Can you work these out from the model? Positions are in its coordinate system, mm. A direction names the side the tool comes from. Give positions to 0.01 mm unless a question says otherwise; leave off trailing zeros. Loops run counter-clockwise (first coordinate to the right, second up) from the corner with the lowest first, then second, coordinate; pieces in that order, holes last. Notation, with made-up numbers: (18, 11) - (53, 11) arc R34 ccw to (53, 43) - close; hole circle Ø7 at (-34.5, 30.5). An arc over 180 degrees is marked (long way). Use a Markdown table: item, result. Add a question column.
```python
from build123d import *

# Parameters (mm, degrees)
BOSS_EXTRUDE1_DEPTH = 348
CUT_EXTRUDE1_DEPTH  = 350


with BuildPart() as part:
    # Sketch1 → Boss-Extrude1 (new body)
    with BuildSketch(Plane.XY):
        Polygon((0, 169.911519959), (-60, 139.911519959), (0, 109.911519959), (60, 139.911519959), align=None)
    extrude(amount=BOSS_EXTRUDE1_DEPTH)

    # Sketch2 → Cut-Extrude1 (cut)
    with BuildSketch(Plane.XY.offset(348)):
        Polygon((48.819660113, 139.911519959), (0, 164.321350015), (-48.819660113, 139.911519959), (0, 115.501689902), align=None)
    extrude(amount=-CUT_EXTRUDE1_DEPTH, mode=Mode.SUBTRACT)


solid = part.part
```
1. Suppose I cut it at A-A (z = 318). List the corners of the cut face in (x, y) for me, and give its area (3 significant figures).
2. Suppose I cut it at C-C (x = 41). List the corners of the cut face in (y, z) for me.
3. If we mould it in two halves opening along Y, with no side actions, what happens to faces 1 (the face through (24.752, 151.946, 176.436)), 2 (the face through (-14, 160, 348)), 3 (the face through (-30.42, 125.12, 171.56)), 4 (the face through (30.42, 154.7, 171.56))? For each: released by +Y, released by -Y, zero draft, split by the parting line, or undercut.
4. Please list where these lines run through material, in increasing order: line 1 along X through (y, z) = (140, 34.5); line 2 along Y through (x, z) = (34.5, 292.5); line 3 along X through (y, z) = (161, 243). Write a range as [from, to].
5. Suppose I cut it at B-B (y = 143.5). List the corners of the cut face in (x, z) for me, and give its area (3 significant figures).
6. Will these pins go through, and if not, where does the flat tip stop? P1, Ø12, axis at y = 159, z = 179.5, coming from the -X side; P2, Ø10, axis at x = 38, y = 148.5, coming from the -Z side; P3, Ø1, axis at x = -4, z = 56.5, coming from the +Y side; P4, Ø1.5, axis at x = -22, z = 226.5, coming from the -Y side.
7. On a 3-axis mill with a long thin cutter (end or side, diameter ignored), from which of +Z, -Z, +X, -X, +Y, -Y can I reach the whole of each face in a straight line? I mean faces 5 (the face through (-14, 160, 0)), 6 (the face through (-24.068, 152.287, 176.436)). Say none if no direction works.
Results below:
| question | item | result |
|---|---|---|
| 1 | outline | (-60, 139.91) - (0, 109.91) - (60, 139.91) - (0, 169.91) - close; hole (-48.82, 139.91) - (0, 115.5) - (48.82, 139.91) - (0, 164.32) - close |
| 1 | area | 1,220 mm² |
| 2 | outline | (130.41, 0) - (136, 0) - (136, 348) - (130.41, 348) - close; (143.82, 0) - (149.41, 0) - (149.41, 348) - (143.82, 348) - close |
| 3 | face 1 | undercut |
| 3 | face 2 | zero draft |
| 3 | face 3 | released by -Y |
| 3 | face 4 | released by +Y |
| 4 | line 1 | [-59.82, -48.64], [48.64, 59.82] |
| 4 | line 2 | [127.16, 132.75], [147.07, 152.66] |
| 4 | line 3 | [-17.82, -6.64], [6.64, 17.82] |
| 5 | outline | (-52.82, 0) - (-41.64, 0) - (-41.64, 348) - (-52.82, 348) - close; (41.64, 0) - (52.82, 0) - (52.82, 348) - (41.64, 348) - close |
| 5 | area | 7,780 mm² |
| 6 | P1 | x = -33.82 |
| 6 | P2 | z = 0 |
| 6 | P3 | y = 168.16 |
| 6 | P4 | y = 120.54 |
| 7 | face 5 | -Z, +X, -X, +Y, -Y |
| 7 | face 6 | +Z, -Z |
